Could you check a few things on this model? Use its own coordinates, in mm. Give positions to 0.01 mm unless a question says otherwise; leave off trailing zeros. Order: outer loops, then holes, each group sorted by start corner. A loop starts at its lowest first (then second) coordinate and runs counter-clockwise, first axis right, second up. Notation, with made-up numbers: (72.25, 19.25) -> (77.25, 19.25) arc R34 ccw to (77.25, 56.25) -> close; hole circle Ø11 at (68, 72.25). An arc over 180 degrees is marked (long way). One line per item, written item: value.
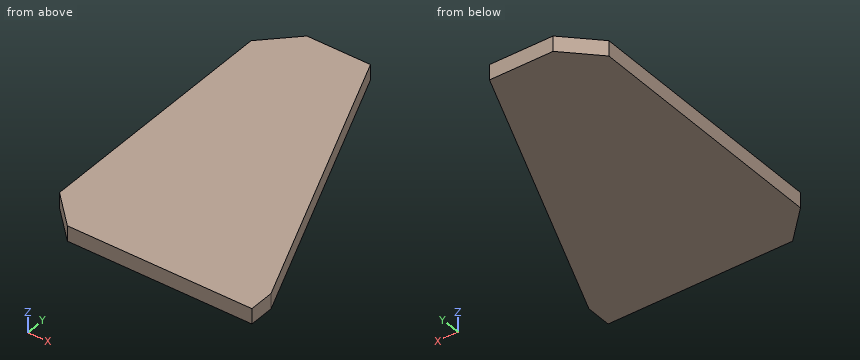
```python
from build123d import *

# Parameters (mm, degrees)
BOSS_EXTRUDE1_DEPTH = 6
CHAMFER1_SIZE       = 25


with BuildPart() as part:
    # Sketch1 → Boss-Extrude1 (new, symmetric)
    with BuildSketch(Plane.XY):
        Polygon((0, 0), (170, 0), (170, 20), (75, 250), (0, 250), align=None)
    extrude(amount=BOSS_EXTRUDE1_DEPTH, both=True)

    # Chamfer1
    chamfer1_edges = [part.edges().sort_by_distance(p)[0] for p in [
        (0, 250, 0),
        (0, 0, 0),
    ]]
    chamfer(chamfer1_edges, length=CHAMFER1_SIZE)


solid = part.part
```
1) Suppose I cut it at B-B, the plane y = 53.5. Write out the boundary of the cut face in (x, z), then the cut area to 3 significant figures.
Answer below:
outline: (0, -6) -> (156.16, -6) -> (156.16, 6) -> (0, 6) -> close
area: 1,870 mm2
2) Suppose I cut it at A-A, the plane z = -3.5. Write out the boundary of the cut face in (x, y).
Answer below:
outline: (0, 25) -> (25, 0) -> (170, 0) -> (170, 20) -> (75, 250) -> (25, 250) -> (0, 225) -> close
3) For P1, Ø3, axis at y = 213, z = -1, coming from the +X side; P2, Ø2, axis at y = 30, z = 2.5, coming from the +X side; P3, Ø6, axis at x = 127, z = 0, coming from the +Y side, each with a flat end and sliding along its axis, tell me the tip position at first contact or that it passes through.
Answer below:
P1: stops at x = 90.9
P2: stops at x = 166.28
P3: stops at y = 131.37
4) Suppose I cut it at C-C, the plane x = 17. Write out the boundary of the cut face in (y, z), then the cut area to 3 significant figures.
Answer below:
outline: (8, -6) -> (242, -6) -> (242, 6) -> (8, 6) -> close
area: 2,810 mm2
5) If I drill on line 1 along X through (y, z) = (152, 0); line 2 along X through (y, z) = (78.5, -5.25); line 3 along Y through (x, z) = (98, -0.25), over which ranges is the centre line in solid material (lowest first)?
Answer below:
line 1: x = 0 to 115.48
line 2: x = 0 to 145.84
line 3: y = 0 to 194.32
